```python
from build123d import *

# Parameters (mm, degrees)
SKETCH1_R           = 60
BOSS_EXTRUDE1_DEPTH = 10


with BuildPart() as part:
    # Sketch1 → Boss-Extrude1 (new body)
    with BuildSketch(Plane.XY):
        with BuildLine():
            Line((-48.3, 63.7), (-48.3, 53.799628252))
            ThreePointArc((-48.3, 53.799628252), (-72.239930825, -2.946590294), (-43.757979913, -57.554575786))
            Line((-43.757979913, -57.554575786), (-42.5, -67.8))
            Line((-42.5, -67.8), (-188.617404673, -85.740961373))
            ThreePointArc((-188.617404673, -85.740961373), (-193.178964964, -86.160109882), (-197.757605429, -86.3))
            Line((-197.757605429, -86.3), (-352.3, -86.3))
            Line((-352.3, -86.3), (-352.3, -54.6))
            Line((-352.3, -54.6), (-306.349572088, -28.070508076))
            ThreePointArc((-306.349572088, -28.070508076), (-296.349572088, -10.75), (-306.349572088, 6.570508076))
            Line((-306.349572088, 6.570508076), (-352.3, 33.1))
            Line((-352.3, 33.1), (-352.3, 63.7))
            Line((-352.3, 63.7), (-48.3, 63.7))
        make_face()
        with Locations((-200, -12)):
            Circle(SKETCH1_R, mode=Mode.SUBTRACT)
    extrude(amount=BOSS_EXTRUDE1_DEPTH)


solid = part.part
```
CAD build for the part. Positions are in the model's coordinates, mm. A direction names the side the tool comes from. Round coordinates to 2 decimals unless told otherwise and drop trailing zeros. Loops run counter-clockwise (first coordinate to the right, second up) from the corner with the lowest first, then second, coordinate; pieces in that order, holes last. Notation, with made-up numbers: M 82,-3 L 90,-3 A15 ccw 90,19 Z; hole C -8.75,58 d8. An arc over 180 degrees is marked long. Return JSON: item names as keys, results as strings. Group by question number.
(1) Mould opens along X. For faces 4 (the cylindrical face through (-259.94, -9.36, 4.93)), 5 (the cylindrical face through (-72.27, -2.06, 4.93)), 6 (the flat face through (-329, 19.65, 4.93)) say: +X half, -X half, draft (parallel to the pull), parting line (faces both ways), or undercut.
(2) Saw through at B-B, the plane y = 20. List the corners of the cut face in (x, z).
(3) Saw through at C-C, the plane x = -214. List the corners of the cut face in (y, z).
(4) Wall check: probe 1 along Y at (x, z) = (-200, 6.75); probe 2 along Y at (x, z) = (-324, 6.5); probe 3 along X at (y, z) = (-27, 4). Give the ranges that are in metal, low to high. Write a range as [from, to].
(5) Tool access for faces 1 (the flat face through (-48.3, 59, 5)), 2 (the cylindrical face through (-193.115, -86.156, 4.93)), 3 (the flat face through (-329.646, -41.521, 4.93)): list every direction of +Z, -Z, +X, -X, +Y, -Y with a clear straight run to the whole face (end or side of a thin tool).
(6) Saw through at A-A, the plane z = 6.5. List the corners of the cut face in (x, y), and give its area (3 significant figures).
(7) Drop flat-ended pins along their axis: P1, Ø1.5, axis at y = -49, z = 2, coming from the -X side; P2, Ø1, axis at y = -55, z = 8.5, coming from the +X side; P3, Ø3, axis at y = -13.5, z = 4, coming from the +X side. Give the stop position or say it passes through.
(8) Saw through at D-D, the plane x = -93. List the corners of the cut face in (y, z), and give its area (3 significant figures).
Answer list:
{
 "1": {"face 4": "undercut", "face 5": "+X half", "face 6": "-X half"},
 "2": {"outline": "M -329.61,0 L -250.75,0 L -250.75,10 L -329.61,10 Z; M -149.25,0 L -69.48,0 L -69.48,10 L -149.25,10 Z"},
 "3": {"outline": "M -86.3,0 L -70.34,0 L -70.34,10 L -86.3,10 Z; M 46.34,0 L 63.7,0 L 63.7,10 L 46.34,10 Z"},
 "4": {"probe 1": "[-86.3, -72], [48, 63.7]", "probe 2": "[-86.3, -38.26], [16.76, 63.7]", "probe 3": "[-304.69, -258.09], [-141.91, -67.07]"},
 "5": {"face 1": "+Z, -Z, +X, +Y", "face 2": "+Z, -Z, +X, -Y", "face 3": "+Z, -Z, -X"},
 "6": {"outline": "M -352.3,-86.3 L -197.76,-86.3 A75 ccw -188.62,-85.74 L -42.5,-67.8 L -43.76,-57.55 A72.3 cw -48.3,53.8 L -48.3,63.7 L -352.3,63.7 L -352.3,33.1 L -306.35,6.57 A20 cw -306.35,-28.07 L -352.3,-54.6 Z; hole C -200,-12 d120", "area": "28,200 mm2"},
 "7": {"P1": "x = -343.9", "P2": "x = -46.34", "P3": "x = -70.73"},
 "8": {"outline": "M -74,0 L 63.7,0 L 63.7,10 L -74,10 Z", "area": "1,380 mm2"}
}
